```python
from build123d import *

# Parameters (mm, degrees)
SKETCH1_R           = 2.75
SKETCH4_R           = 2.4
BOSS_EXTRUDE1_DEPTH = 1
SKETCH5_R           = 2.7531
BOSS_EXTRUDE2_DEPTH = 31
CHAMFER2_SIZE       = 2
CHAMFER2_SIZE2      = 1.154700538
CHAMFER3_SIZE       = 0.5


with BuildPart() as part:
    # Sweep1: sweep along a path in Sketch2
    with BuildLine(Plane(origin=(0, 0, 0), x_dir=(1, 0, 0), z_dir=(0, 1, 0))) as sweep1_path:
        Line((0, 0), (0, 48.343145751))
        ThreePointArc((0, 48.343145751), (0.30448187, 49.87387948), (1.171572875, 51.171572875))
        Line((1.171572875, 51.171572875), (12.02081528, 62.02081528))
    # Sketch1 → Sweep1 (sweep)
    with BuildSketch(Plane.XY):
        Circle(SKETCH1_R)
    sweep(path=sweep1_path.line)

    # Sketch4 → Boss-Extrude1 (add)
    with BuildSketch(Plane.XY):
        Circle(SKETCH4_R)
    extrude(amount=BOSS_EXTRUDE1_DEPTH)

    # Sketch5 → Boss-Extrude2 (add)
    with BuildSketch(Plane.XY.offset(1)):
        with Locations((-0.271402, 0)):
            Circle(SKETCH5_R)
    extrude(amount=BOSS_EXTRUDE2_DEPTH)

    # Chamfer2
    chamfer2_edges = [part.edges().sort_by_distance(p)[0] for p in [
        (-3.024502, 0, 32),
    ]]
    chamfer2_side = [part.faces().sort_by_distance(p)[0] for p in [
        (-3.024502, 0, 16.5),
    ]]
    chamfer(chamfer2_edges, length=CHAMFER2_SIZE, length2=CHAMFER2_SIZE2, reference=chamfer2_side[0])

    # Chamfer3
    chamfer3_edges = [part.edges().sort_by_distance(p)[0] for p in [
        (10.076271632, 0, -63.965358928),
    ]]
    chamfer(chamfer3_edges, length=CHAMFER3_SIZE)


solid = part.part
```
Geometry check sheet. Reference: the model listing, model coordinates, mm. A direction names the side the tool comes from. Round coordinates to 2 decimals unless told otherwise and drop trailing zeros. Loops run counter-clockwise (first coordinate to the right, second up) from the corner with the lowest first, then second, coordinate; pieces in that order, holes last. Notation, with made-up numbers: M -20.5,66 L 17.5,66 A26 ccw 17.5,84 Z; hole C 67.5,83.25 d2. An arc over 180 degrees is marked long. Return JSON: item names as keys, results as strings. Group by question number.
(1) Set-up check for faces 1 (the face through (0, 0, 32)), 2 (the face through (-0.596, 2.685, -24.51)): record each of +Z, -Z, +X, -X, +Y, -Y from which the full face is reachable in a straight line by a thin tool's end or side.
(2) Section check B-B, the plane z = 8. Enter the section's corners in (x, y), and give its area (3 significant figures).
(3) Section check C-C, the plane z = -42. Enter the section's corners in (x, y).
(4) Scan lines: line 1 along X through (y, z) = (0.25, 6.5); line 2 along Z through (x, y) = (6.25, -1.1); line 3 along X through (y, z) = (2.3, -9). Record each from-to range of solid material in increasing order. Write a range as [from, to].
(5) Section check A-A, the plane y = 0. Enter the section's corners in (x, z), and give its area (3 significant figures).
(6) Mould release check, pull along Z, two halves, no side actions. Record for faces 3 (the face through (2.272, -1.054, 15.297)), 4 (the face through (12.04, -0.03, -62)), 5 (the face through (-2.53, -0.4, 1)), 6 (the face through (1.29, 2.024, 0.493)): pulls with the +Z half, pulls with the -Z half, needs draft (parallel to the pull), parting line crosses it, or undercut.
(7) Go/stop test with flat-tipped pins: pin 1 (1.7 mm diameter, centred on x = 0.5, y = -0.5, fed in from -Z); pin 2 (3 mm diameter, centred on x = 7, y = -0.5, fed in from +Z); pin 3 (1 mm diameter, centred on x = 0.5, z = 1, fed in from -Y). Record where each tip stops, or that it passes through.
Data:
{
 "1": {"face 1": "+Z, +X, -X, +Y, -Y", "face 2": "none"},
 "2": {"outline": "C -0.27,0 d5.51", "area": "23.8 mm²"},
 "3": {"outline": "C 0,0 d5.5"},
 "4": {"line 1": "[-3.01, 2.47]", "line 2": "[-59.81, -52.69]", "line 3": "[-1.51, 1.51]"},
 "5": {"outline": "M -3.02,1 L -2.4,1 L -2.4,0 L -2.75,0 L -2.75,-48.34 A6.75 ccw -0.77,-53.12 L 9.72,-63.61 L 10.43,-63.61 L 13.61,-60.43 L 13.61,-59.72 L 3.12,-49.23 A1.25 cw 2.75,-48.34 L 2.75,0 L 2.4,0 L 2.4,1 L 2.48,1 L 2.48,30 L 1.33,32 L -1.87,32 L -3.02,30 Z", "area": "540 mm²"},
 "6": {"face 3": "needs draft", "face 4": "pulls with the -Z half", "face 5": "undercut", "face 6": "undercut"},
 "7": {"pin 1": "z = -55.19", "pin 2": "z = -51.65", "pin 3": "y = -2.74"}
}
